```python
from build123d import *

# Parameters (mm, degrees)
SKETCH1_W              = 30
SKETCH1_H              = 6.5
BOSS_EXTRUDE1_DEPTH    = 9.5
SKETCH2_R              = 2
CUT_EXTRUDE1_DEPTH     = 19.907670401
M3_TAPPED_HOLE1_REACH  = 20.05
M3_TAPPED_HOLE1_BORE_R = 1.25
CHAMFER1_SIZE          = 0.5


with BuildPart() as part:
    # Sketch1 → Boss-Extrude1 (new body)
    with BuildSketch(Plane.XY):
        Rectangle(SKETCH1_W, SKETCH1_H)
    extrude(amount=BOSS_EXTRUDE1_DEPTH)

    # Sketch2 → Cut-Extrude1 (cut, through all)
    with BuildSketch(Plane(origin=(0, 3.25, 0), x_dir=(1, 0, 0), z_dir=(0, 1, 0))):
        with Locations(Location((-12, -5.5, 0), (0, 0, 180))):
            Circle(SKETCH2_R)
        with Locations(Location((12, -5.5, 0), (0, 0, 180))):
            Circle(SKETCH2_R)
    extrude(amount=-CUT_EXTRUDE1_DEPTH, mode=Mode.SUBTRACT)

    # M3 Tapped Hole1 bore → M3 Tapped Hole1 (cut, up to next)
    with BuildSketch(Plane(origin=(0, 0, 0), x_dir=(-1, 0, 0), z_dir=(0, 0, -1)), mode=Mode.PRIVATE) as m3_tapped_hole1_sk1:
        with Locations((12, 0)):
            Circle(M3_TAPPED_HOLE1_BORE_R)
    m3_tapped_hole1_tool1 = extrude(m3_tapped_hole1_sk1.sketch, amount=-M3_TAPPED_HOLE1_REACH, mode=Mode.PRIVATE) & part.part
    # M3 Tapped Hole1 bore → M3 Tapped Hole1 (cut, up to next)
    with BuildSketch(Plane(origin=(0, 0, 0), x_dir=(-1, 0, 0), z_dir=(0, 0, -1)), mode=Mode.PRIVATE) as m3_tapped_hole1_sk2:
        with Locations((-12, 0)):
            Circle(M3_TAPPED_HOLE1_BORE_R)
    m3_tapped_hole1_tool2 = extrude(m3_tapped_hole1_sk2.sketch, amount=-M3_TAPPED_HOLE1_REACH, mode=Mode.PRIVATE) & part.part
    add(m3_tapped_hole1_tool1.solids().sort_by_distance((-12, 0, 0))[0], mode=Mode.SUBTRACT)
    add(m3_tapped_hole1_tool2.solids().sort_by_distance((12, 0, 0))[0], mode=Mode.SUBTRACT)

    # Chamfer1
    chamfer1_edges = [part.edges().sort_by_distance(p)[0] for p in [
        (0, 3.25, 9.5),
        (0, 3.25, 0),
        (0, -3.25, 0),
        (0, -3.25, 9.5),
    ]]
    chamfer(chamfer1_edges, length=CHAMFER1_SIZE)


solid = part.part
```
Geometry check sheet. Reference: the model listing, model coordinates, mm. A direction names the side the tool comes from. Coordinates: 2 decimals unless noted, no trailing zeros. Loops run counter-clockwise (first coordinate to the right, second up) from the corner with the lowest first, then second, coordinate; pieces in that order, holes last. Notation, with made-up numbers: (84.5, -31.5) -> (130.5, -31.5) arc R19 ccw to (130.5, -9.5) -> close; hole circle Ø2 at (63, 24). An arc over 180 degrees is marked (long way). Put each result on its own line as item: value.
1) Cross-section at A-A on z = 5. Record the boundary of the cut face in (x, y).
Result set:
outline: (-15, -3.25) -> (-13.94, -3.25) -> (-13.94, 3.25) -> (-15, 3.25) -> close; (-10.06, -3.25) -> (10.06, -3.25) -> (10.06, 3.25) -> (-10.06, 3.25) -> close; (13.94, -3.25) -> (15, -3.25) -> (15, 3.25) -> (13.94, 3.25) -> close
2) Tool access check on faces 1 (the cylindrical face through (13.25, 0.05, 1.94)), 2 (the flat face through (0, 0, 9.5)). Record the directions out of +Z, -Z, +X, -X, +Y, -Y that give a thin tool (end or side, any length) a straight path to the whole face; none if there is none.
Result set:
face 1: -Z
face 2: +Z, +X, -X, +Y, -Y
3) Cross-section at B-B on x = 12. Record the boundary of the cut face in (y, z).
Result set:
outline: (-3.25, 0.5) -> (-2.75, 0) -> (-1.25, 0) -> (-1.25, 3.5) -> (-3.25, 3.5) -> close; (-3.25, 7.5) -> (3.25, 7.5) -> (3.25, 9) -> (2.75, 9.5) -> (-2.75, 9.5) -> (-3.25, 9) -> close; (1.25, 0) -> (2.75, 0) -> (3.25, 0.5) -> (3.25, 3.5) -> (1.25, 3.5) -> close
4) Gauge pin test, flat ends, axial feed: pin 1 Ø3 at (x, z) = (-12, 5.5) entering from +Y; pin 2 Ø3 at (x, z) = (11.5, 4.5) entering from -Y. Record the tip position at first contact, or that the pin passes through.
Result set:
pin 1: passes through
pin 2: stops at y = -3.25
5) Thickness scan on line 1 (X direction, y = 0, z = 2.55); line 2 (Y direction, x = -12, z = 1.2); line 3 (Z direction, x = -12, y = 1.5). Record the ranges inside material, lowest first.
Result set:
line 1: x = -15 to -13.25, -10.75 to 10.75, 13.25 to 15
line 2: y = -3.25 to -1.25, 1.25 to 3.25
line 3: z = 0 to 3.5, 7.5 to 9.5
6) Release check for a two-part mould opening along X. For faces 3 (the flat face through (-15, 0, 5)), 4 (the flat face through (15, 0, 5)), 5 (the flat face through (0, 0, 0)), 6 (the cylindrical face through (12.26, 0.046, 7.483)) record: released by +X, released by -X, zero draft, split by the parting line, or undercut.
Result set:
face 3: released by -X
face 4: released by +X
face 5: zero draft
face 6: undercut
7) Cross-section at C-C on y = -1.75. Record the boundary of the cut face in (x, z).
Result set:
outline: (-15, 0) -> (15, 0) -> (15, 9.5) -> (-15, 9.5) -> close; hole circle Ø4 at (-12, 5.5); hole circle Ø4 at (12, 5.5)
8) Cross-section at D-D on y = 0. Record the boundary of the cut face in (x, z).
Result set:
outline: (-15, 0) -> (-13.25, 0) -> (-13.25, 3.94) arc R2 cw (long way) to (-10.75, 3.94) -> (-10.75, 0) -> (10.75, 0) -> (10.75, 3.94) arc R2 cw (long way) to (13.25, 3.94) -> (13.25, 0) -> (15, 0) -> (15, 9.5) -> (-15, 9.5) -> close
